Read the model definition and answer for the solid it produces. Units are mm, in the model's axes. A direction names the side the tool comes from. Give positions to 0.01 mm unless a question says otherwise; leave off trailing zeros. Write each loop counter-clockwise with the first axis right and the second up, starting at its lowest first coordinate (ties: lowest second). Pieces come first, ordered by that corner, then holes. Notation, with made-up numbers: (70, 23.25) - (106, 23.25) arc R16 ccw to (106, 33.25) - close; hole circle Ø2 at (-18.5, 6.5). An arc over 180 degrees is marked (long way). Answer as CSV lines item,"result".
```python
from build123d import *

# Parameters (mm, degrees)
CHAMFER1_SIZE = 0.5


with BuildPart() as part:
    # Sketch1 → Revolve1 (revolve)
    with BuildSketch(Plane.XY):
        Polygon((695.508784709, 32.474610335), (685.508784709, 32.474610335), (685.508784709, 34.849610335), (681.508784709, 34.849610335), (681.508784709, 42.349610335), (598.508784709, 42.349610335), (598.508784709, 37.349610335), (591.508784709, 37.349610335), (591.508784709, 27.349610335), (695.508784709, 27.349610335), align=None)
    revolve(axis=Axis((695.508784709, 27.349610335, 0), (-1, 0, 0)))

    # Chamfer1
    chamfer1_edges = [part.edges().sort_by_distance(p)[0] for p in [
        (598.508784709, 12.349610335, 0),
        (591.508784709, 17.349610335, 0),
        (695.508784709, 22.224610335, 0),
        (685.508784709, 19.849610335, 0),
        (681.508784709, 12.349610335, 0),
    ]]
    chamfer(chamfer1_edges, length=CHAMFER1_SIZE)


solid = part.part
```
(1) Each of these flat-tipped pins is pushed along its axis until it touches: P1, Ø1.5, axis at x = 637.5, y = 31, coming from the +Z side; P2, Ø5, axis at x = 616, y = 37.5, coming from the -Z side; P3, Ø6, axis at x = 655.5, z = 12, coming from the -Y side. Where does it stop, or does it pass through?
Worked out:
P1,"stops at z = 14.72"
P2,"stops at z = -12.9"
P3,"stops at y = 15.35"
(2) For faces 1 (the flat face through (598.509, 17, 3)), 2 (the flat face through (681.509, 21, 6)), 3 (the flat face through (695.509, 27, 0)), determine the directions among +Z, -Z, +X, -X, +Y, -Y from which every point of the face is accessible in a straight line to the end or side of a thin tool.
Worked out:
face 1,"-X"
face 2,"+X"
face 3,"+Z, -Z, +X, +Y, -Y"
(3) A cutting plane is placed at B-B (x = 601). Write down the section's boundary in (y, z), and give its area (3 significant figures).
Worked out:
outline,"circle Ø30 at (27.35, 0)"
area,"707 mm^2"
(4) A cutting plane is placed at A-A (z = 0). Write down the section's boundary in (x, y), and give its area (3 significant figures).
Worked out:
outline,"(591.51, 17.85) - (592.01, 17.35) - (598.51, 17.35) - (598.51, 12.85) - (599.01, 12.35) - (681.01, 12.35) - (681.51, 12.85) - (681.51, 19.85) - (685.01, 19.85) - (685.51, 20.35) - (685.51, 22.22) - (695.01, 22.22) - (695.51, 22.72) - (695.51, 31.97) - (695.01, 32.47) - (685.51, 32.47) - (685.51, 34.35) - (685.01, 34.85) - (681.51, 34.85) - (681.51, 41.85) - (681.01, 42.35) - (599.01, 42.35) - (598.51, 41.85) - (598.51, 37.35) - (592.01, 37.35) - (591.51, 36.85) - close"
area,"2,790 mm^2"
(5) Find the intervals of material crossed by L1, parallel to Y at x = 620, z = -13; L2, parallel to X at y = 25.5, z = -8.25; L3, parallel to X at y = 14.5, z = 6.75, in increasing order.
Worked out:
L1,"y = 19.87 to 34.83"
L2,"x = 591.51 to 681.51"
L3,"x = 598.52 to 681.49"
